Can you work these out from the model? Positions are in its coordinate system, mm. A direction names the side the tool comes from. Round coordinates to 2 decimals unless told otherwise and drop trailing zeros. Loops run counter-clockwise (first coordinate to the right, second up) from the corner with the lowest first, then second, coordinate; pieces in that order, holes last. Notation, with made-up numbers: (74, 64) -> (79, 64) arc R29 cw to (79, 85) -> close; hole circle Ø10 at (81, 37). An arc over 180 degrees is marked (long way). Write item = value, one per line.
from build123d import *

# Parameters (mm, degrees)
BOSS_EXTRUDE1_START = 13.904652831
SKETCH2_R           = 3
BOSS_EXTRUDE1_DEPTH = 13.904652831
BOSS_EXTRUDE2_DEPTH = 5
SKETCH4_R           = 2.15
BOSS_EXTRUDE3_DEPTH = 7
CHAMFER1_SIZE       = 0.2
CHAMFER2_SIZE       = 0.3


with BuildPart() as part:
    # Sketch1 → Revolve1 (revolve)
    with BuildSketch(Plane(origin=(0, 0, 0), x_dir=(-1, 0, 0), z_dir=(0, 0, -1)), mode=Mode.PRIVATE) as revolve1_sk:
        Polygon((-4, -29.495347169), (0, -29.495347169), (0, 5.1), (-4, 5.1), (-4, -10.6), (-3, -10.6), (-3, -11.6), (-4, -11.6), align=None)
    revolve(revolve1_sk.sketch.rotate(Axis((0, -29.495347169, 0), (0, 1, 0)), 270), axis=Axis((0, -29.495347169, 0), (0, 1, 0)))

    # Sketch2 → Boss-Extrude1 (add)
    with BuildSketch(Plane.XZ.offset(29.495347169).offset(BOSS_EXTRUDE1_START)):
        with Locations(Location((0, 0, 0), (0, 0, 90))):
            Circle(SKETCH2_R)
    extrude(amount=-BOSS_EXTRUDE1_DEPTH)

    # Sketch3 → Boss-Extrude2 (add)
    with BuildSketch(Plane(origin=(0, 5.1, 0), x_dir=(-1, 0, 0), z_dir=(0, 1, 0))):
        with BuildLine():
            Line((3.417793986, -0.754111574), (0.754142944, -3.417787065))
            ThreePointArc((0.754142944, -3.417787065), (1.6062e-05, -3.5), (-0.754111574, -3.417793986))
            Line((-0.754111574, -3.417793986), (-3.417787065, -0.754142944))
            ThreePointArc((-3.417787065, -0.754142944), (-3.5, -1.6062e-05), (-3.417793986, 0.754111574))
            Line((-3.417793986, 0.754111574), (-0.754142944, 3.417787065))
            ThreePointArc((-0.754142944, 3.417787065), (0, 3.5), (0.754142944, 3.417787065))
            Line((0.754142944, 3.417787065), (3.417787065, 0.754142944))
            ThreePointArc((3.417787065, 0.754142944), (3.5, 1.6062e-05), (3.417793986, -0.754111574))
        make_face()
    extrude(amount=BOSS_EXTRUDE2_DEPTH)

    # Sketch4 → Boss-Extrude3 (add)
    with BuildSketch(Plane(origin=(0, 10.1, 0), x_dir=(-1, 0, 0), z_dir=(0, 1, 0))):
        with Locations(Location((0, 0, 0), (0, 0, 90))):
            Circle(SKETCH4_R)
    extrude(amount=BOSS_EXTRUDE3_DEPTH)

    # Chamfer1
    chamfer1_edges = [part.edges().sort_by_distance(p)[0] for p in [
        (0, -29.495347169, -4),
        (0, 5.1, -4),
    ]]
    chamfer(chamfer1_edges, length=CHAMFER1_SIZE)

    # Chamfer2
    chamfer2_edges = [part.edges().sort_by_distance(p)[0] for p in [
        (0, -43.4, -3),
    ]]
    chamfer(chamfer2_edges, length=CHAMFER2_SIZE)


solid = part.part
1. Suppose I cut it at C-C, the plane y = -26.5. List the corners of the cut face in (x, z) for me.
Entries:
outline = circle Ø8 at (0, 0)
2. For faces 4 (the cylindrical face through (-1.308, 13.551, -1.706)), 5 (the flat face through (3, -10.6, 1)), 6 (the flat face through (-2.07, 7.56, 2.1)), 7 (the cylindrical face through (0, 7.6, 3.5)), 8 (the flat face through (2.1, 7.56, 2.07)), which set-ups out of +Z, -Z, +X, -X, +Y, -Y let a thin tool reach every point of the face, with its end or its side?
Entries:
face_4 = +Y
face_5 = none
face_6 = +Z, -X, +Y
face_7 = +Z, +Y
face_8 = +Z, +X, +Y
3. I need wall thicknesses on line 1 (Y direction, x = 0.5, z = -3.5); line 2 (Y direction, x = -0.5, z = -3); line 3 (X direction, y = -15, z = 1.25). Which ranges of each line are inside material? Lowest first, please. Write a range as [from, to].
Entries:
line_1 = [-29.5, -11.6], [-10.6, 5.1]
line_2 = [-29.5, -11.6], [-10.6, 10.1]
line_3 = [-3.8, 3.8]
4. I'm going to push flat-ended pins straight in: pin 1 (3 mm diameter, centred on x = -0.5, z = -3, fed in from -Y); pin 2 (2 mm diameter, centred on y = -32.5, z = 1, fed in from -X); pin 3 (1 mm diameter, centred on y = 2.5, z = -3, fed in from -X); pin 4 (2 mm diameter, centred on y = -25.5, z = -3, fed in from +X). Where does each tip first touch, or does it pass through?
Entries:
pin_1 = -43.4
pin_2 = -3
pin_3 = -3.12
pin_4 = 3.46
5. We'd pull the mould along Y, two halves only. Please class faces 1 (the cylindrical face through (-0.9, -36.39, 2.86)), 2 (the cylindrical face through (0.9, -11.11, 2.86)), 3 (the flat face through (0, 10.1, 2.4)): released by +Y, released by -Y, zero draft, split by the parting line, or undercut.
Entries:
face_1 = zero draft
face_2 = undercut
face_3 = released by +Y
